Check sheet for the modelled part. Datum: model origin and axes. Units: mm. Give positions to 0.01 mm unless a question says otherwise; leave off trailing zeros. Write each loop counter-clockwise with the first axis right and the second up, starting at its lowest first coordinate (ties: lowest second). Pieces come first, ordered by that corner, then holes. Notation, with made-up numbers: (-16.5, 57.5) -> (14.5, 57.5) arc R34 ccw to (14.5, 87.5) -> close; hole circle Ø1 at (-8, 5). An arc over 180 degrees is marked (long way). Return JSON: item names as keys, results as strings.
from build123d import *

# Parameters (mm, degrees)
EXTRUDE_575_DEPTH   = 12
SKETCH_4_OUTSIDE_W  = 93.598
SKETCH_4_OUTSIDE_H  = 96.382
SKETCH_4_OUTSIDE_R  = 9
CUT_EXTRUDE_1_DEPTH = 19.248287591
CUT_EXTRUDE_1_DRAFT = -60
SKETCH_5_OUTSIDE_W  = 117.332
SKETCH_5_OUTSIDE_H  = 120.116
SKETCH_5_OUTSIDE_R  = 9
CUT_EXTRUDE_2_DEPTH = 26.099800796
CUT_EXTRUDE_2_DRAFT = -60
SKETCH_6_R          = 5.188125
CUT_EXTRUDE_3_DEPTH = 10


with BuildPart() as part:
    # 草图1 → Extrude 575 (new body)
    with BuildSketch(Plane.XY):
        Polygon((0, 10.392304845), (-9, 5.196152423), (-9, -5.196152423), (0, -10.392304845), (9, -5.196152423), (9, 5.196152423), align=None)
    extrude(amount=EXTRUDE_575_DEPTH)

    # 草图2 → 凸台-旋转1 (revolve)
    with BuildSketch(Plane(origin=(0, 0, 0), x_dir=(1, 0, 0), z_dir=(0, 1, 0))):
        with BuildLine():
            Line((0, 9), (0, 0))
            Line((0, 0), (9, 0))
            ThreePointArc((9, 0), (6.363961031, 6.363961031), (0, 9))
        make_face()
    revolve(axis=Axis((0, 0, -2.579649935), (0, 0, 1)))


with BuildPart() as cut_extrude_1_tool:
    # 草图4 outside → 切除-拉伸1 (with draft: the straight prism first)
    with BuildSketch(Plane(origin=(0, 0, 0), x_dir=(-1, 0, 0), z_dir=(0, 0, -1))):
        Rectangle(SKETCH_4_OUTSIDE_W, SKETCH_4_OUTSIDE_H)
        Circle(SKETCH_4_OUTSIDE_R, mode=Mode.SUBTRACT)
    extrude(amount=-CUT_EXTRUDE_1_DEPTH)
    # 切除-拉伸1: the draft: its side faces are tilted about the plane it starts from
    cut_extrude_1_sides = [cut_extrude_1_tool.faces().sort_by_distance(p)[0] for p in [
        (0, -48.191, 9.624143795),
        (-46.799, 0, 9.624143795),
        (0, 48.191, 9.624143795),
        (46.799, 0, 9.624143795),
        (9, 0, 9.624143795),
    ]]
    draft(cut_extrude_1_sides, Plane(origin=(0, 0, 0), x_dir=(-1, 0, 0), z_dir=(0, 0, -1)), CUT_EXTRUDE_1_DRAFT)


with BuildPart() as part_1:
    add(part.part)

    # 切除-拉伸1: cut by cut_extrude_1_tool
    add(cut_extrude_1_tool.part, mode=Mode.SUBTRACT)


with BuildPart() as cut_extrude_2_tool:
    # 草图5 outside → 切除-拉伸2 (with draft: the straight prism first)
    with BuildSketch(Plane.XY.offset(12)):
        Rectangle(SKETCH_5_OUTSIDE_W, SKETCH_5_OUTSIDE_H)
        Circle(SKETCH_5_OUTSIDE_R, mode=Mode.SUBTRACT)
    extrude(amount=-CUT_EXTRUDE_2_DEPTH)
    # 切除-拉伸2: the draft: its side faces are tilted about the plane it starts from
    cut_extrude_2_sides = [cut_extrude_2_tool.faces().sort_by_distance(p)[0] for p in [
        (0, -60.058, -1.049900398),
        (58.666, 0, -1.049900398),
        (0, 60.058, -1.049900398),
        (-58.666, 0, -1.049900398),
        (-9, 0, -1.049900398),
    ]]
    draft(cut_extrude_2_sides, Plane.XY.offset(12), CUT_EXTRUDE_2_DRAFT)


with BuildPart() as part_2:
    add(part_1.part)

    # 切除-拉伸2: cut by cut_extrude_2_tool
    add(cut_extrude_2_tool.part, mode=Mode.SUBTRACT)

    # 草图6 → 切除-拉伸3 (cut)
    with BuildSketch(Plane.XY.offset(12)):
        Circle(SKETCH_6_R)
    extrude(amount=-CUT_EXTRUDE_3_DEPTH, mode=Mode.SUBTRACT)


solid = part_2.part
(1) Depth check by flat-ended pin: pin 1 Ø1 at (y, z) = (1.5, -1) entering from +X; pin 2 Ø10 at (x, z) = (7, 9) entering from -Y; pin 3 Ø3 at (x, y) = (2, -1.5) entering from +Z. Enter the tip coordinate at first touch or a pass-through.
Reply:
{"pin 1": "x = 8.91", "pin 2": "y = -9.24", "pin 3": "z = 2"}
(2) Thickness scan on L1, parallel to Y at x = -4, z = 7; L2, parallel to X at y = 3.25, z = 3.75; L3, parallel to Y at x = -2.5, z = 7. Record the ranges inside material, lowest first.
Reply:
{"L1": "-8.08 to -3.3, 3.3 to 8.08", "L2": "-9 to -4.04, 4.04 to 9", "L3": "-8.95 to -4.55, 4.55 to 8.95"}
(3) Release check for a two-part mould opening along X. For faces 1 (the cylindrical face through (4.95, 1.56, 7.07)), 2 (the conical face through (8.09, -4.65, 0.19)), 3 (the flat face through (4, -4, 12)) record: pulls with the +X half, pulls with the -X half, needs draft (parallel to the pull), parting line crosses it, or undercut.
Reply:
{"face 1": "undercut", "face 2": "pulls with the +X half", "face 3": "needs draft"}
(4) Cross-section at A-A on z = 7.75. Enter the section's corners in (x, y).
Reply:
{"outline": "(-9, -5.2) -> (0, -10.39) -> (9, -5.2) -> (9, 5.2) -> (0, 10.39) -> (-9, 5.2) -> close; hole circle Ø10.38 at (0, 0)"}
